The figure shows three views and two pictorial views of one solid part (mm, origin at its lowest corner). Answer the questions. Round coordinates to 2 decimals unless told otherwise and drop trailing zeros. Order: outer loops, then holes, each group sorted by start corner. A loop starts at its lowest first (then second) coordinate and runs counter-clockwise, first axis right, second up. Notation, with made-up numbers: (-10, 12.5) - (-2, 12.5) arc R21 ccw to (-2, 28.5) - close; hole circle Ø9 at (32, -18.75). An arc over 180 degrees is marked (long way). Use CSV: the item, a comma, the result in double quotes.
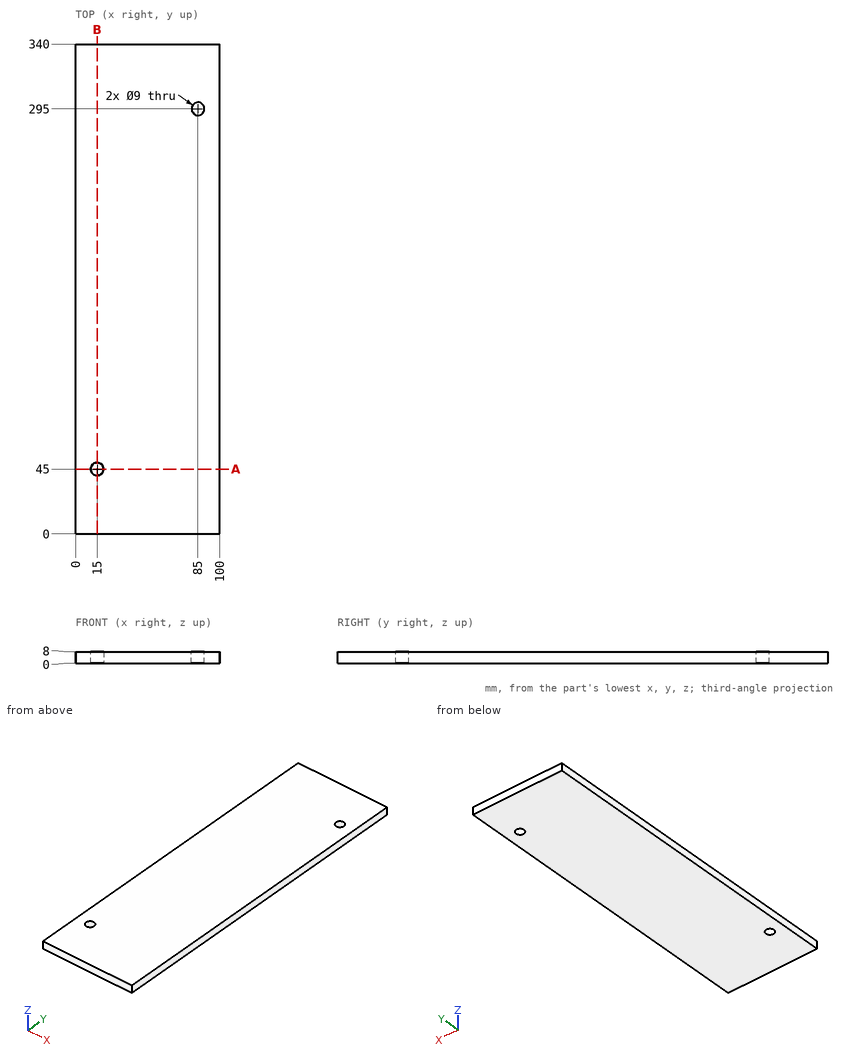
(1) Find section A-A (y = 45). Determine the outline of the cut face in (x, z).
Findings below:
outline,"(0, 0) - (10.5, 0) - (10.5, 8) - (0, 8) - close; (19.5, 0) - (100, 0) - (100, 8) - (19.5, 8) - close"
(2) Find the intervals of material crossed by L1, parallel to X at y = 295, z = 5.75; L2, parallel to X at y = 45, z = 6; L3, parallel to Y at x = 85, z = 4.5, in increasing order. Write a range as from..to.
Findings below:
L1,"x = 0..80.5, 89.5..100"
L2,"x = 0..10.5, 19.5..100"
L3,"y = 0..290.5, 299.5..340"
(3) Each of these flat-tipped pins is pushed along its axis until it touches: pin 1 (1 mm diameter, centred on x = 55, z = 5, fed in from -Y); pin 2 (8 mm diameter, centred on x = 85, y = 295, fed in from +Z). Where does it stop, or does it pass through?
Findings below:
pin 1,"stops at y = 0"
pin 2,"passes through"
(4) Find section B-B (x = 15). Determine the outline of the cut face in (y, z).
Findings below:
outline,"(0, 0) - (40.5, 0) - (40.5, 8) - (0, 8) - close; (49.5, 0) - (340, 0) - (340, 8) - (49.5, 8) - close"
